Study the drawing (mm; zero at the part's minimum x, y, z) and answer. A direction names the side the tool comes from. Coordinates: 2 decimals unless noted, no trailing zeros. Loops run counter-clockwise (first coordinate to the right, second up) from the corner with the lowest first, then second, coordinate; pieces in that order, holes last. Notation, with made-up numbers: (57, 75) - (62, 75) arc R12 ccw to (62, 97) - close; hole circle Ø10 at (13, -16). An arc over 180 degrees is marked (long way). Use one line per item in the form item = value.
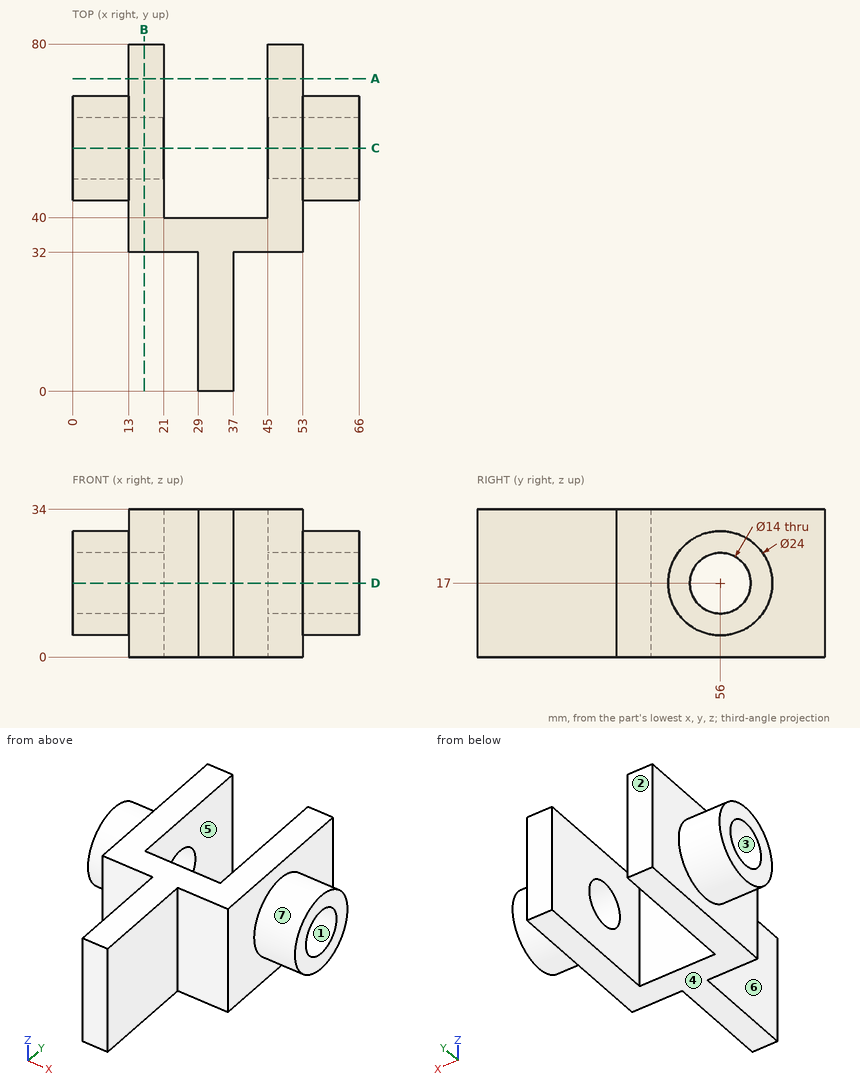
Item 1: The part is cut by section C-C on y = 56. Give the vertices of the cut face in (x, z), plus the area to 3 significant figures.
Results below:
outline = (0, 5) - (13, 5) - (13, 0) - (21, 0) - (21, 10) - (0, 10) - close; (0, 24) - (21, 24) - (21, 34) - (13, 34) - (13, 29) - (0, 29) - close; (45, 0) - (53, 0) - (53, 5) - (66, 5) - (66, 10) - (45, 10) - close; (45, 24) - (66, 24) - (66, 29) - (53, 29) - (53, 34) - (45, 34) - close
area = 580 mm²
Item 2: Find the intervals of material crossed by L1, parallel to X at y = 49, z = 28; L2, parallel to X at y = 54.5, z = 8.5; L3, parallel to Z at x = 6.75, y = 56, in increasing order.
Results below:
L1 = 13 to 21, 45 to 53
L2 = 0 to 21, 45 to 66
L3 = 5 to 10, 24 to 29
Item 3: For a pull along Z with two mould halves and no side action, classify the marked faces 1, 2, 3 and 4 as +Z half, -Z half, draft (parallel to the pull), parting line (faces both ways), or undercut.
Results below:
face_1 = undercut
face_2 = draft
face_3 = undercut
face_4 = -Z half
Item 4: The part is cut by section A-A on y = 72. Give the vertices of the cut face in (x, z), plus the area to 3 significant figures.
Results below:
outline = (13, 0) - (21, 0) - (21, 34) - (13, 34) - close; (45, 0) - (53, 0) - (53, 34) - (45, 34) - close
area = 544 mm²
Item 5: Each of these flat-tipped pins is pushed along its axis until it touches: P1, Ø5, axis at x = 47.5, z = 12, coming from the -Y side; P2, Ø1, axis at x = 8.5, z = 17.5, coming from the -Y side; P3, Ø7, axis at x = 36, z = 16.5, coming from the +Y side. Where does it stop, or does it pass through?
Results below:
P1 = 32
P2 = 44
P3 = 40
Item 6: The part is cut by section B-B on x = 16.5. Give the vertices of the cut face in (y, z), plus the area to 3 significant figures.
Results below:
outline = (32, 0) - (80, 0) - (80, 34) - (32, 34) - close; hole circle Ø14 at (56, 17)
area = 1,480 mm²
Item 7: The part is cut by section D-D on z = 17. Give the vertices of the cut face in (x, y).
Results below:
outline = (0, 44) - (13, 44) - (13, 32) - (29, 32) - (29, 0) - (37, 0) - (37, 32) - (53, 32) - (53, 44) - (66, 44) - (66, 49) - (45, 49) - (45, 40) - (21, 40) - (21, 49) - (0, 49) - close; (0, 63) - (21, 63) - (21, 80) - (13, 80) - (13, 68) - (0, 68) - close; (45, 63) - (66, 63) - (66, 68) - (53, 68) - (53, 80) - (45, 80) - close
Item 8: Which of the six approach directions +Z, -Z, +X, -X, +Y, -Y give full straight-line access (tool end or side, diameter ignored) to the marked faces 5, 6 and 7?
Results below:
face_5 = +Z, -Z, +Y
face_6 = +Z, -Z, -X, -Y
face_7 = +X
